Input: part model. Units: mm. Frame: model coordinates. Face numbers are marked on the shaded views. A direction names the side the tool comes from. Coordinates: 2 decimals unless noted, no trailing zeros. Write each loop counter-clockwise with the first axis right and the second up, starting at its lowest first coordinate (ties: lowest second). Pieces come first, ordered by that corner, then holes. Notation, with made-up numbers: M 19,10 L 30,10 A34 cw 30,48 Z; hole C 36,89.25 d10. An arc over 180 degrees is marked long. Use one line per item in the form item = value.
from build123d import *

# Parameters (mm, degrees)
SKETCH_1_W          = 65
SKETCH_1_H          = 60
EXTRUDE_1_DEPTH     = 12
SKETCH_4_W          = 45
SKETCH_4_H          = 16
EXTRUDE_2_DEPTH     = 12
SKETCH_5_W          = 42
SKETCH_5_H          = 76
CUT_EXTRUDE_1_DEPTH = 1.5
HOLE_WIZARD_M4_1_D  = 3.3


with BuildPart() as part:
    # 草图1 → 凸台-拉伸1 (new body)
    with BuildSketch(Plane.XY):
        Rectangle(SKETCH_1_W, SKETCH_1_H)
    extrude(amount=EXTRUDE_1_DEPTH)

    # 草图4 → 凸台-拉伸2 (add)
    with BuildSketch(Plane(origin=(0, 0, 0), x_dir=(-1, 0, 0), z_dir=(0, 0, -1))):
        with Locations((10, 38)):
            Rectangle(SKETCH_4_W, SKETCH_4_H)
    extrude(amount=-EXTRUDE_2_DEPTH)

    # 草图5 → 切除-拉伸1 (cut)
    with BuildSketch(Plane(origin=(0, 0, 0), x_dir=(-1, 0, 0), z_dir=(0, 0, -1))):
        with Locations((11.5, 8)):
            Rectangle(SKETCH_5_W, SKETCH_5_H)
    extrude(amount=-CUT_EXTRUDE_1_DEPTH, mode=Mode.SUBTRACT)

    # M4 螺纹孔1 (through all)
    with Locations(Plane(origin=(-10, 42, 12), x_dir=(1, 0, 0), z_dir=(0, 0, 1))):
        with Locations((0, 0)):
            Hole(HOLE_WIZARD_M4_1_D / 2)


solid = part.part
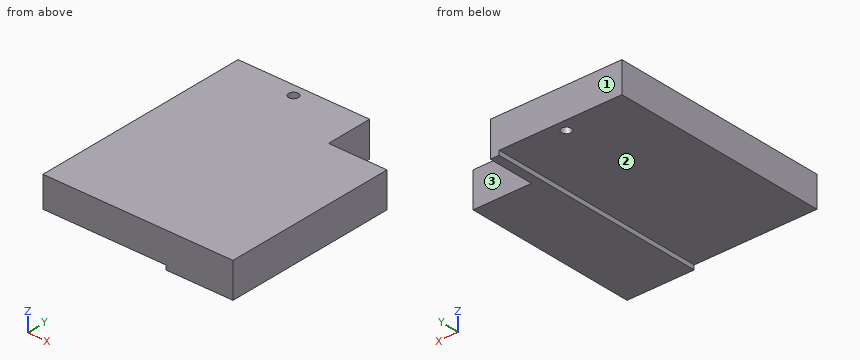
(1) Section query D-D on y = -21. Return the cut outline in (x, z).
Computed:
outline = M -32.5,1.5 L 9.5,1.5 L 9.5,0 L 32.5,0 L 32.5,12 L -32.5,12 Z
(2) Line query: probe 1 along Y at (x, z) = (-10, 6.5); probe 2 along X at (y, z) = (41.5, 7); probe 3 along X at (y, z) = (-26, 1). Output: solid intervals per line, ascending.
Computed:
probe_1 = -30 to 40.35, 43.65 to 46
probe_2 = -32.5 to -11.57, -8.43 to 12.5
probe_3 = 9.5 to 32.5
(3) Section query B-B on y = 42. Return the cut outline in (x, z), plus the area to 3 significant figures.
Computed:
outline = M -32.5,1.5 L -11.65,1.5 L -11.65,12 L -32.5,12 Z; M -8.35,1.5 L 9.5,1.5 L 9.5,0 L 12.5,0 L 12.5,12 L -8.35,12 Z
area = 442 mm^2
(4) Set-up query: the marked faces 1, 2 and 3. Return all of +Z, -Z, +X, -X, +Y, -Y with unobstructed straight access to the full face (end or side cutting, diameter ignored); none if empty.
Computed:
face_1 = +Z, -Z, +X, -X, +Y
face_2 = -Z, -X, +Y, -Y
face_3 = +Z, -Z, +X, +Y
(5) Section query A-A on x = -10. Return the cut outline in (y, z).
Computed:
outline = M -30,1.5 L 40.35,1.5 L 40.35,12 L -30,12 Z; M 43.65,1.5 L 46,1.5 L 46,12 L 43.65,12 Z
(6) First-contact query: pin 1 Ø6 at (x, z) = (22, 4.5) entering from +Y; pin 2 Ø21 at (x, y) = (-19, 26.5) entering from -Z; pin 3 Ø3 at (x, y) = (-10, 42) entering from +Z; pin 4 Ø0.8 at (y, z) = (3.5, 1) entering from -X. Flat tips, straight axial feed; report the tip coordinate or a pass-through.
Computed:
pin_1 = 30
pin_2 = 1.5
pin_3 = through
pin_4 = 9.5
(7) Section query C-C on z = 5. Return the cut outline in (x, y).
Computed:
outline = M -32.5,-30 L 32.5,-30 L 32.5,30 L 12.5,30 L 12.5,46 L -32.5,46 Z; hole C -10,42 d3.3
